Check sheet for the modelled part. Datum: model origin and axes. Units: mm. Face numbers are marked on the shaded views. Round coordinates to 2 decimals unless told otherwise and drop trailing zeros. Order: outer loops, then holes, each group sorted by start corner. A loop starts at its lowest first (then second) coordinate and runs counter-clockwise, first axis right, second up. Notation, with made-up numbers: (25, 23.25) -> (33, 23.25) arc R26 cw to (33, 43.25) -> close; hole circle Ø10 at (64.25, 57). An arc over 180 degrees is marked (long way). Answer in a Markdown table with one row per item.
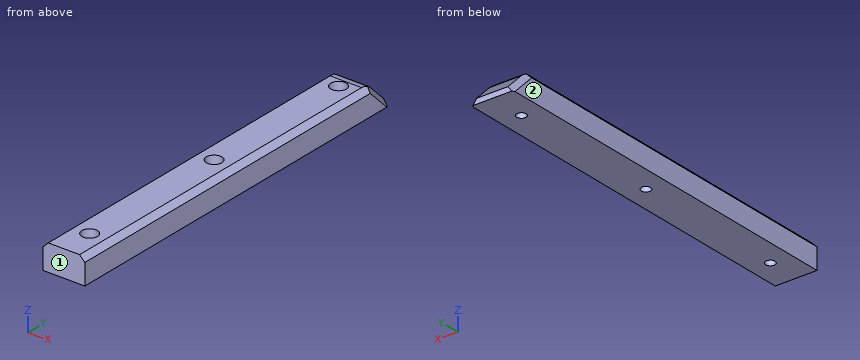
```python
from build123d import *

# Parameters (mm, degrees)
SKETCH1_W                                          = 40
SKETCH1_H                                          = 366
BOSS_EXTRUDE1_DEPTH                                = 25
CHAMFER2_SIZE                                      = 20
SKETCH4_R                                          = 7.5
CUT_EXTRUDE1_DEPTH                                 = 2
HOLE_SIZE_BASED_ON_HEX_SOCKET_CAP_SCRE_D           = 9
HOLE_SIZE_BASED_ON_HEX_SOCKET_CAP_SCRE_CBORE_D     = 15
HOLE_SIZE_BASED_ON_HEX_SOCKET_CAP_SCRE_CBORE_DEPTH = 10
CHAMFER3_SIZE                                      = 5
CHAMFER4_SIZE                                      = 5
FILLET4_R                                          = 15


with BuildPart() as part:
    # Sketch1 → Boss-Extrude1 (new body)
    with BuildSketch(Plane.XY):
        Rectangle(SKETCH1_W, SKETCH1_H)
    extrude(amount=BOSS_EXTRUDE1_DEPTH)

    # Chamfer2
    chamfer2_edges = [part.edges().sort_by_distance(p)[0] for p in [
        (0, 183, 25),
    ]]
    chamfer(chamfer2_edges, length=CHAMFER2_SIZE)

    # Sketch4 → Cut-Extrude1 (cut)
    with BuildSketch(Plane.XY.offset(25)):
        with Locations((0, -152)):
            Circle(SKETCH4_R)
        with Locations((0, -2)):
            Circle(SKETCH4_R)
        with Locations((0, 148)):
            Circle(SKETCH4_R)
    extrude(amount=-CUT_EXTRUDE1_DEPTH, mode=Mode.SUBTRACT)

    # Hole Size (based on) hex socket cap screw type 1 (through all)
    with Locations(Plane.XY.offset(23)):
        with Locations((0, -152), (0, -2), (0, 148)):
            CounterBoreHole(HOLE_SIZE_BASED_ON_HEX_SOCKET_CAP_SCRE_D / 2, HOLE_SIZE_BASED_ON_HEX_SOCKET_CAP_SCRE_CBORE_D / 2, HOLE_SIZE_BASED_ON_HEX_SOCKET_CAP_SCRE_CBORE_DEPTH)

    # Chamfer3
    chamfer3_edges = [part.edges().sort_by_distance(p)[0] for p in [
        (-20, -10, 25),
        (20, -10, 25),
    ]]
    chamfer(chamfer3_edges, length=CHAMFER3_SIZE)

    # Chamfer4
    chamfer4_edges = [part.edges().sort_by_distance(p)[0] for p in [
        (20, 175.5, 12.5),
        (-20, 175.5, 12.5),
    ]]
    chamfer(chamfer4_edges, length=CHAMFER4_SIZE)

    # Fillet4
    fillet4_edges = [part.edges().sort_by_distance(p)[0] for p in [
        (0, 163, 25),
    ]]
    fillet(fillet4_edges, radius=FILLET4_R)


solid = part.part
```
(1) Draft check along Y on the marked faces 1 and 2. Enter one of: pulls with the +Y half, pulls with the -Y half, needs draft (parallel to the pull), parting line crosses it, or undercut.
Solutions:
| item | result |
|---|---|
| face 1 | pulls with the -Y half |
| face 2 | needs draft |
(2) Scan lines: probe 1 along Y at (x, z) = (0, 3); probe 2 along Y at (x, z) = (0, 15.5); probe 3 along X at (y, z) = (-151, 19.5). Record each from-to range of solid material in increasing order. Write a range as from..to.
Solutions:
| item | result |
|---|---|
| probe 1 | -183..-156.5, -147.5..-6.5, 2.5..143.5, 152.5..183 |
| probe 2 | -183..-159.5, -144.5..-9.5, 5.5..140.5, 155.5..172.5 |
| probe 3 | -20..-7.43, 7.43..20 |
(3) Depth check by flat-ended pin: pin 1 Ø4 at (x, z) = (-12.5, 18.5) entering from +Y; pin 2 Ø7.5 at (x, y) = (-1, -152) entering from +Z; pin 3 Ø1 at (x, z) = (-15.5, 8) entering from +Y. Enter the tip coordinate at first touch or a pass-through.
Solutions:
| item | result |
|---|---|
| pin 1 | y = 171.5 |
| pin 2 | z = 13 |
| pin 3 | y = 180.16 |
(4) Section check A-A on x = 0. Give the number of separate pieces and of enclosed holes in the cut face, plus the area to 3 significant figures.
Solutions:
| item | result |
|---|---|
| separate pieces | 4 |
| enclosed holes | 0 |
| area | 8,050 mm^2 |
(5) Section check C-C on y = 104. Record the boundary of the cut face in (x, z), plus the area to 3 significant figures.
Solutions:
| item | result |
|---|---|
| outline | (-20, 0) -> (20, 0) -> (20, 20) -> (15, 25) -> (-15, 25) -> (-20, 20) -> close |
| area | 975 mm^2 |
(6) Section check B-B on y = -152. Record the boundary of the cut face in (x, z), plus the area to 3 significant figures.
Solutions:
| item | result |
|---|---|
| outline | (-20, 0) -> (-4.5, 0) -> (-4.5, 13) -> (-7.5, 13) -> (-7.5, 25) -> (-15, 25) -> (-20, 20) -> close; (4.5, 0) -> (20, 0) -> (20, 20) -> (15, 25) -> (7.5, 25) -> (7.5, 13) -> (4.5, 13) -> close |
| area | 678 mm^2 |
